Could you check a few things on this model? Use its own coordinates, in mm. A direction names the side the tool comes from. Coordinates: 2 decimals unless noted, no trailing zeros. Order: outer loops, then holes, each group sorted by start corner. A loop starts at its lowest first (then second) coordinate and runs counter-clockwise, first axis right, second up. Notation, with made-up numbers: (28.5, 87.25) - (57.5, 87.25) arc R19 ccw to (57.5, 113.25) - close; hole circle Ø5 at (-19.75, -3.5). An arc over 180 degrees is marked (long way). One line per item, written item: value.
from build123d import *

# Parameters (mm, degrees)
SKETCH1_W               = 96.012
SKETCH1_H               = 15.875
BASE_EXTRUDE_DEPTH      = 7.9375
CUT_EXTRUDE1_DEPTH      = 98.638740648
FILLET5_R               = 0.635
FILLET6_R               = 3.81
FILLET7_R               = 3.175
FILLET8_R               = 6.35
FILLET9_R               = 6.35
FILLET10_R              = 6.35
BOSS_EXTRUDE3_START     = -6.35
BOSS_EXTRUDE3_DEPTH     = 6.35
FILLET11_R              = 3.81
SKETCH7_R               = 2.54
CUT_EXTRUDE5_DEPTH      = 99.512406834
CUT_EXTRUDE6_DEPTH      = 99.485470295
CUT_EXTRUDE6_DEPTH_BACK = 99.485470295
SKETCH8_W               = 56.651025612
SKETCH8_H               = 0.0254
FILLET12_R              = 3.81
FILLET13_R              = 3.81


with BuildPart() as part:
    # Sketch1 → Base-Extrude (new, symmetric)
    with BuildSketch(Plane.XY):
        with Locations((48.006, 7.9375)):
            Rectangle(SKETCH1_W, SKETCH1_H)
    extrude(amount=BASE_EXTRUDE_DEPTH, both=True)

    # Sketch3 → Cut-Extrude1 (cut, through all)
    with BuildSketch(Plane(origin=(0, 15.875, 0), x_dir=(-1, 0, 0), z_dir=(0, 1, 0))):
        Polygon((-53.213, -4.7625), (-92.837, -4.7625), (-92.837, 4.7625), (-53.213, 4.7625), (-48.4505, 0), align=None)
        Polygon((2.11806403, -3.175), (-47.135371939, -3.175), (-55.848364541, -11.887992602), (2.11806403, -11.887992602), align=None)
        Polygon((2.11806403, 3.175), (-47.135371939, 3.175), (-55.848364541, 11.887992602), (2.11806403, 11.887992602), align=None)
    extrude(amount=-CUT_EXTRUDE1_DEPTH, mode=Mode.SUBTRACT)

    # Fillet5
    fillet5_edges = [part.edges().sort_by_distance(p)[0] for p in [
        (53.213, 7.9375, -4.7625),
        (53.213, 7.9375, 4.7625),
        (47.135371939, 7.9375, 3.175),
        (47.135371939, 7.9375, -3.175),
    ]]
    fillet(fillet5_edges, radius=FILLET5_R)

    # Fillet6
    fillet6_edges = [part.edges().sort_by_distance(p)[0] for p in [
        (51.897871939, 7.9375, 7.9375),
        (51.897871939, 7.9375, -7.9375),
    ]]
    fillet(fillet6_edges, radius=FILLET6_R)

    # Fillet7
    fillet7_edges = [part.edges().sort_by_distance(p)[0] for p in [
        (92.837, 7.9375, -4.7625),
        (92.837, 7.9375, 4.7625),
    ]]
    fillet(fillet7_edges, radius=FILLET7_R)

    # Fillet8
    fillet8_edges = [part.edges().sort_by_distance(p)[0] for p in [
        (96.012, 7.9375, 7.9375),
        (96.012, 7.9375, -7.9375),
    ]]
    fillet(fillet8_edges, radius=FILLET8_R)

    # Fillet9
    fillet9_edges = [part.edges().sort_by_distance(p)[0] for p in [
        (0, 15.875, 0),
    ]]
    fillet(fillet9_edges, radius=FILLET9_R)

    # Fillet10
    fillet10_edges = [part.edges().sort_by_distance(p)[0] for p in [
        (0, 0, 0),
    ]]
    fillet(fillet10_edges, radius=FILLET10_R)

    # Sketch6 → Boss-Extrude3 (add)
    with BuildSketch(Plane.XY.offset(3.175).offset(BOSS_EXTRUDE3_START)):
        with BuildLine():
            Line((5.564108911, 15.826180461), (30.825163366, 18.976770691))
            ThreePointArc((30.825163366, 18.976770691), (39.943880119, 14.786551928), (40.249024971, 4.755808431))
            ThreePointArc((40.249024971, 4.755808431), (36.72434383, -2.446073762), (28.949130797, -4.404784191))
            Line((28.949130797, -4.404784191), (5.165376283, 0.111477206))
            ThreePointArc((5.165376283, 0.111477206), (1.458943846, 2.300300048), (0, 6.35))
            Line((0, 6.35), (0, 9.525))
            ThreePointArc((0, 9.525), (1.590120358, 13.728099546), (5.564108911, 15.826180461))
        make_face()
    extrude(amount=BOSS_EXTRUDE3_DEPTH)

    # Fillet11
    fillet11_edges = [part.edges().sort_by_distance(p)[0] for p in [
        (38.862, 0, 0),
        (39.103515829, 15.875, 0),
    ]]
    fillet(fillet11_edges, radius=FILLET11_R)

    # Sketch7 → Cut-Extrude5 (cut, through all)
    with BuildSketch(Plane.XY.offset(3.175)):
        with Locations((6.35, 9.525)):
            Circle(SKETCH7_R)
        with Locations((32.004, 9.525)):
            Circle(SKETCH7_R)
    extrude(amount=-CUT_EXTRUDE5_DEPTH, mode=Mode.SUBTRACT)

    # Sketch8 → Cut-Extrude6 (cut, two sides: drawn at the far end of the back side and taken through both)
    with BuildSketch(Plane(origin=(0, 15.875, 0), x_dir=(-1, 0, 0), z_dir=(0, 1, 0)).offset(-CUT_EXTRUDE6_DEPTH_BACK)):
        with Locations((-25.150512806, 0)):
            Rectangle(SKETCH8_W, SKETCH8_H)
    extrude(amount=CUT_EXTRUDE6_DEPTH + CUT_EXTRUDE6_DEPTH_BACK, mode=Mode.SUBTRACT)

    # Fillet12
    fillet12_edges = [part.edges().sort_by_distance(p)[0] for p in [
        (48.4632, 7.9375, 0.0127),
    ]]
    fillet(fillet12_edges, radius=FILLET12_R)

    # Fillet13
    fillet13_edges = [part.edges().sort_by_distance(p)[0] for p in [
        (48.4632, 7.9375, -0.0127),
    ]]
    fillet(fillet13_edges, radius=FILLET13_R)


solid = part.part
Item 1: Thinking about a two-plate mould opening in Z: for faces 4 (the face through (33.906, -4.026, 1.572)), 5 (the face through (48.36, 7.83, -0.31)), 6 (the face through (71, 8, -4.762)), 7 (the face through (71, 8, -7.938)), which applies, pulls with the +Z half, pulls with the -Z half, needs draft (parallel to the pull), parting line crosses it, or undercut?
Conclusion:
face 4: needs draft
face 5: undercut
face 6: undercut
face 7: pulls with the -Z half
Item 2: I'm going to push flat-ended pins straight in: pin 1 Ø4 at (y, z) = (2.5, -1.5) entering from -X; pin 2 Ø6 at (x, y) = (6.35, 9.525) entering from -Z (3 decimals); pin 3 Ø7 at (x, y) = (25.5, 12.5) entering from +Z (3 decimals). Where does each tip first touch, or does it pass through?
Conclusion:
pin 1: x = 0.28
pin 2: z = -3.175
pin 3: z = 3.175
Item 3: If I drill on probe 1 along X at (y, z) = (11, -3); probe 2 along Z at (x, y) = (55, 4.5); probe 3 along Y at (x, z) = (91, -6) (3 decimals), over which ranges is the centre line in solid material (lowest first)?
Conclusion:
probe 1: 0.17 to 4.28, 8.42 to 29.94, 34.07 to 51.45, 92.51 to 95.85
probe 2: -7.94 to -4.76, 4.76 to 7.94
probe 3: 0 to 15.875
Item 4: I want a section at D-D on x = 20. Please give me the cut outline in (y, z) (3 decimals).
Conclusion:
outline: (-2.705, -3.175) - (17.627, -3.175) - (17.627, -0.013) - (-2.705, -0.013) - close; (-2.705, 0.013) - (17.627, 0.013) - (17.627, 3.175) - (-2.705, 3.175) - close
Item 5: For faces 1 (the face through (24, 7, -3.175)), 2 (the face through (1.55, 13.68, 1.57)), 3 (the face through (51.33, 8.05, 2.88)), which set-ups out of +Z, -Z, +X, -X, +Y, -Y let a thin tool reach every point of the face, with its end or its side?
Conclusion:
face 1: -Z, -X, +Y, -Y
face 2: +Z, -Z, -X, +Y
face 3: +Y, -Y
Item 6: I want a section at A-A on x = 70. Please give me the cut outline in (y, z) (1 decimal), then the cut area to 3 significant figures.
Conclusion:
outline: (0, -7.9) - (15.9, -7.9) - (15.9, -4.8) - (0, -4.8) - close; (0, 4.8) - (15.9, 4.8) - (15.9, 7.9) - (0, 7.9) - close
area: 101 mm²
Item 7: I want a section at B-B on x = 33. Please give me the cut outline in (y, z) (3 decimals), then the cut area to 3 significant figures.
Conclusion:
outline: (-4.297, -3.175) - (7.188, -3.175) - (7.188, -0.013) - (-4.297, -0.013) - close; (-4.297, 0.013) - (7.188, 0.013) - (7.188, 3.175) - (-4.297, 3.175) - close; (11.862, -3.175) - (18.998, -3.175) - (18.998, -0.013) - (11.862, -0.013) - close; (11.862, 0.013) - (18.998, 0.013) - (18.998, 3.175) - (11.862, 3.175) - close
area: 118 mm²
